Source: CAD feature listing. Evaluate the final solid. Frame: model axes, mm. A direction names the side the tool comes from. Give positions to 0.01 mm unless a question says otherwise; leave off trailing zeros. Order: outer loops, then holes, each group sorted by start corner. A loop starts at its lowest first (then second) coordinate and runs counter-clockwise, first axis right, second up. Notation, with made-up numbers: M -29,14 L -2,14 A32 ccw -2,48 Z; hole C 1,1 d4. An arc over 180 degrees is marked long. Answer as a JSON object with one key per item and string values. Group by question number.
1. Section query B-B (x = -35). Output: boundary loops of the cut face in (y, z), plus the area to 3 significant figures.
2. Section query D-D (y = 0). Count the separate pieces of the cut face and the enclosed holes in it, plus the area to 3 significant figures.
3. Section query A-A (y = 9). Output: boundary loops of the cut face in (x, z).
4. Pin query (flat end, axial travel): P1, Ø3, axis at x = 34.5, y = -20.5, coming from the -Z side; P2, Ø3, axis at x = -24.5, y = -1.5, coming from the +Z side; P3, Ø6, axis at x = -22.5, z = -19.5, coming from the +Y side; P4, Ø7, axis at x = -36.5, z = -4, coming from the +Y side. Return the tip coordinate at first contact, or that it passes through.
5. Set-up query: faces 5 (the flat face through (-26, 0, -29)), 6 (the flat face through (-40, 0, -33)), 7 (the flat face through (-32, -18, -19)). Return all of +Z, -Z, +X, -X, +Y, -Y with unobstructed straight access to the full face (end or side cutting, diameter ignored); none if empty.
6. Section query C-C (z = -15.5). Output: boundary loops of the cut face in (x, y), plus the area to 3 significant figures.
7. Material intervals for L1, parallel to X at y = 0, z = -35; L2, parallel to Z at x = -34, y = 6.5; L3, parallel to Y at x = 25.5, z = -15, sorted ascending. Write a range as [from, to].
8. Pull-direction query (Y, two-part tool) for faces 1 (the flat face through (-1, -18, -38)), 2 (the flat face through (33, -4, -33)), 3 (the flat face through (-34, -4, -4)), 4 (the flat face through (32, -18, -19)); classes: +Y half, -Y half, draft (parallel to the pull), parting line (faces both ways), or undercut.
from build123d import *

# Parameters (mm, degrees)
BODY_PROFILE_SKETCH_R       = 17
BODY_PROFILE_SKETCH_W       = 13
BODY_PROFILE_SKETCH_H       = 8
BODY_EXTRUDE_38MM_DEPTH     = 38
WINDOW_CUT_20X14_DEPTH      = 100.584135283
WINDOW_CUT_20X14_DEPTH_BACK = 100.584135283
WINDOW_20X14_SKETCH_W       = 20
WINDOW_20X14_SKETCH_H       = 14
WINDOW_CUT_18X20_DEPTH      = 74.518705103
WINDOW_CUT_18X20_DEPTH_BACK = 74.518705103
WINDOW_18X20_SKETCH_W       = 18
WINDOW_18X20_SKETCH_H       = 20


with BuildPart() as part:
    # Body Profile Sketch → Body Extrude 38mm (new body)
    with BuildSketch(Plane.XY):
        with BuildLine():
            Line((-44, -18), (-20.124611797, -18))
            ThreePointArc((-20.124611797, -18), (0, -27), (20.124611797, -18))
            Line((20.124611797, -18), (44, -18))
            Line((44, -18), (44, 18))
            Line((44, 18), (20.124611797, 18))
            ThreePointArc((20.124611797, 18), (0, 27), (-20.124611797, 18))
            Line((-20.124611797, 18), (-44, 18))
            Line((-44, 18), (-44, -18))
        make_face()
        Circle(BODY_PROFILE_SKETCH_R, mode=Mode.SUBTRACT)
        with Locations((-33.5, 0)):
            Rectangle(BODY_PROFILE_SKETCH_W, BODY_PROFILE_SKETCH_H, mode=Mode.SUBTRACT)
        with Locations((33.5, 0)):
            Rectangle(BODY_PROFILE_SKETCH_W, BODY_PROFILE_SKETCH_H, mode=Mode.SUBTRACT)
    extrude(amount=-BODY_EXTRUDE_38MM_DEPTH)

    # Window 20x14 Sketch → Window Cut 20x14 (cut, two sides: drawn at the far end of the back side and taken through both)
    with BuildSketch(Plane.ZY.offset(44).offset(-WINDOW_CUT_20X14_DEPTH_BACK)):
        with Locations((-19, 0)):
            Rectangle(WINDOW_20X14_SKETCH_W, WINDOW_20X14_SKETCH_H)
    extrude(amount=WINDOW_CUT_20X14_DEPTH + WINDOW_CUT_20X14_DEPTH_BACK, mode=Mode.SUBTRACT)

    # Window 18x20 Sketch → Window Cut 18x20 (cut, two sides: drawn at the far end of the back side and taken through both)
    with BuildSketch(Plane(origin=(0, 18, 0), x_dir=(1, 0, 0), z_dir=(0, 1, 0)).offset(-WINDOW_CUT_18X20_DEPTH_BACK)):
        with Locations((0, 19)):
            Rectangle(WINDOW_18X20_SKETCH_W, WINDOW_18X20_SKETCH_H)
    extrude(amount=WINDOW_CUT_18X20_DEPTH + WINDOW_CUT_18X20_DEPTH_BACK, mode=Mode.SUBTRACT)


solid = part.part
Answer sheet:
{
 "1": {"outline": "M -18,-38 L -4,-38 L -4,-29 L -7,-29 L -7,-9 L -4,-9 L -4,0 L -18,0 Z; M 4,-38 L 18,-38 L 18,0 L 4,0 L 4,-9 L 7,-9 L 7,-29 L 4,-29 Z", "area": "944 mm^2"},
 "2": {"separate pieces": "8", "enclosed holes": "0", "area": "504 mm^2"},
 "3": {"outline": "M -44,-38 L -14.42,-38 L -14.42,0 L -44,0 Z; M 14.42,-38 L 44,-38 L 44,0 L 14.42,0 Z"},
 "4": {"P1": "through", "P2": "z = 0", "P3": "y = 18.67", "P4": "y = 18"},
 "5": {"face 5": "+X, -X", "face 6": "+Z, -Z", "face 7": "+Z, -Z, -X, -Y"},
 "6": {"outline": "M -44,-18 L -20.12,-18 A27 ccw -9,-25.46 L -9,-14.42 A17 cw -15.49,-7 L -44,-7 Z; M -44,7 L -15.49,7 A17 cw -9,14.42 L -9,25.46 A27 ccw -20.12,18 L -44,18 Z; M 9,-25.46 A27 ccw 20.12,-18 L 44,-18 L 44,-7 L 15.49,-7 A17 cw 9,-14.42 Z; M 9,14.42 A17 cw 15.49,7 L 44,7 L 44,18 L 20.12,18 A27 ccw 9,25.46 Z", "area": "1,620 mm^2"},
 "7": {"L1": "[-44, -40], [-27, -17], [17, 27], [40, 44]", "L2": "[-38, -29], [-9, 0]", "L3": "[-18, -7], [7, 18]"},
 "8": {"face 1": "draft", "face 2": "undercut", "face 3": "undercut", "face 4": "-Y half"}
}
